```python
from build123d import *

# Parameters (mm, degrees)
BASE_BLOCK_DEPTH       = 42
TOP_BOSS_SKETCH_W      = 30
TOP_BOSS_SKETCH_H      = 30
TOP_BOSS_30X30_DEPTH   = 20
VERTICAL_BORE_SKETCH_R = 10
VERTICAL_BORE_DEPTH    = 98.693397935
CROSS_HOLE_SKETCH_R    = 6
CROSS_HOLE_DEPTH       = 75.759614766
ANGLED_POCKET_DEPTH    = 94.61448679
ARCH_CUTOUT_DEPTH      = 98.693397984
ARCH_CUTOUT_DEPTH_BACK = 98.693397984


with BuildPart() as part:
    # Base Block Profile Sketch → Base Block (new body)
    with BuildSketch(Plane.XY):
        Polygon((0, 0), (74, 0), (74, 28), (34, 28), (0, 20), align=None)
    extrude(amount=BASE_BLOCK_DEPTH)

    # Top Boss Sketch → Top Boss 30x30 (add)
    with BuildSketch(Plane(origin=(0, 28, 0), x_dir=(1, 0, 0), z_dir=(0, 1, 0))):
        with Locations((54, -21)):
            Rectangle(TOP_BOSS_SKETCH_W, TOP_BOSS_SKETCH_H)
    extrude(amount=TOP_BOSS_30X30_DEPTH)

    # Vertical Bore Sketch → Vertical Bore (cut, through all)
    with BuildSketch(Plane(origin=(0, 48, 0), x_dir=(1, 0, 0), z_dir=(0, 1, 0))):
        with Locations(Location((54, -21, 0), (0, 0, 180))):
            Circle(VERTICAL_BORE_SKETCH_R)
    extrude(amount=-VERTICAL_BORE_DEPTH, mode=Mode.SUBTRACT)

    # Cross Hole Sketch → Cross Hole (cut, through all)
    with BuildSketch(Plane.ZY.offset(-39)):
        with Locations((21, 38)):
            Circle(CROSS_HOLE_SKETCH_R)
    extrude(amount=-CROSS_HOLE_DEPTH, mode=Mode.SUBTRACT)

    # Angled Pocket Sketch → Angled Pocket (cut, through all)
    with BuildSketch(Plane(origin=(-4.459016393, 18.950819672, 0), x_dir=(0.973417168333576, 0.22903933372554744, 0), z_dir=(-0.22903933372554744, 0.973417168333576, 0))):
        Polygon((11.580786675, -21), (11.580786675, -15), (31.580786675, -15), (31.580786675, -27), (11.580786675, -27), align=None)
    extrude(amount=-ANGLED_POCKET_DEPTH, mode=Mode.SUBTRACT)

    # Arch Cutout Sketch → Arch Cutout (cut, two sides: drawn at the far end of the back side and taken through both)
    with BuildSketch(Plane.ZY.offset(-ARCH_CUTOUT_DEPTH_BACK)):
        with BuildLine():
            Line((36, -130.00000016), (36, 0))
            ThreePointArc((36, 0), (21, 15), (6, 0))
            Line((6, 0), (6, -130.00000016))
            Line((6, -130.00000016), (6, -390.00000048))
            Line((6, -390.00000048), (36, -390.00000048))
            Line((36, -390.00000048), (36, -130.00000016))
        make_face()
    extrude(amount=ARCH_CUTOUT_DEPTH + ARCH_CUTOUT_DEPTH_BACK, mode=Mode.SUBTRACT)


solid = part.part
```
Build history of the part. All positions in model axes, mm. A direction names the side the tool comes from. Round coordinates to 2 decimals unless told otherwise and drop trailing zeros. Order: outer loops, then holes, each group sorted by start corner. A loop starts at its lowest first (then second) coordinate and runs counter-clockwise, first axis right, second up. Notation, with made-up numbers: (48.5, -26) - (59.5, -26) arc R20 ccw to (59.5, -15) - close; hole circle Ø1 at (-17.5, 42.25). An arc over 180 degrees is marked (long way). Use a Markdown table: item, result.
1) Tool access for faces 1 (the face through (54, 38, 36)), 2 (the face through (69, 38, 28)), 3 (the face through (27.725, 20.053, 20.916)), 4 (the face through (7.725, 17.73, 20.916)): list every direction of +Z, -Z, +X, -X, +Y, -Y with a clear straight run to the whole face (end or side of a thin tool).
Recorded:
| item | result |
|---|---|
| face 1 | +Z, +X, -X, +Y |
| face 2 | +Z, -Z, +X, +Y |
| face 3 | -Y |
| face 4 | +Y |
2) Saw through at D-D on x = 65. Write the cut outline in (y, z).
Recorded:
| item | result |
|---|---|
| outline | (0, 0) - (28, 0) - (28, 6) - (48, 6) - (48, 36) - (28, 36) - (28, 42) - (0, 42) - (0, 36) arc R15 cw to (0, 6) - close; hole circle Ø12 at (38, 21) |
3) Wall check: L1, parallel to Y at x = 67, z = 21; L2, parallel to Z at x = 66.25, y = 38; L3, parallel to Z at x = 54, y = 27. Give the ranges that are in metal, low to high.
Recorded:
| item | result |
|---|---|
| L1 | y = 15 to 32, 44 to 48 |
| L2 | z = 6 to 15, 27 to 36 |
| L3 | z = 0 to 11, 31 to 42 |
4) Pull direction Z, two halves, no side cores. Call faces 5 (the face through (39, 38, 28)), 6 (the face through (41.67, 35.7, 26.54)), 7 (the face through (54, 38, 6)): pulls with the +Z half, pulls with the -Z half, needs draft (parallel to the pull), parting line crosses it, or undercut.
Recorded:
| item | result |
|---|---|
| face 5 | needs draft |
| face 6 | undercut |
| face 7 | pulls with the -Z half |
5) Saw through at B-B on y = 38. Write the cut outline in (x, z), and give its area (3 significant figures).
Recorded:
| item | result |
|---|---|
| outline | (39, 6) - (69, 6) - (69, 15) - (62, 15) arc R10 cw to (46, 15) - (39, 15) - close; (39, 27) - (46, 27) arc R10 cw to (62, 27) - (69, 27) - (69, 36) - (39, 36) - close |
| area | 451 mm² |
6) Saw through at A-A on x = 54. Write the cut outline in (y, z), and give its area (3 significant figures).
Recorded:
| item | result |
|---|---|
| outline | (0, 0) - (28, 0) - (28, 6) - (48, 6) - (48, 11) - (11.18, 11) arc R15 cw to (0, 6) - close; (0, 36) arc R15 cw to (11.18, 31) - (48, 31) - (48, 36) - (28, 36) - (28, 42) - (0, 42) - close |
| area | 739 mm² |
7) Saw through at C-C on z = 14. Write the cut outline in (x, y).
Recorded:
| item | result |
|---|---|
| outline | (0, 13.27) - (46.86, 13.27) - (46.86, 48) - (39, 48) - (39, 28) - (34, 28) - (0, 20) - close; (61.14, 13.27) - (74, 13.27) - (74, 28) - (69, 28) - (69, 48) - (61.14, 48) - close |
8) Flat gauge pins, fed straight in: pin 1 Ø7 at (y, z) = (38, 21) entering from +X; pin 2 Ø12 at (y, z) = (40.5, 35) entering from +X; pin 3 Ø2 at (x, z) = (40.5, 14) entering from -Y; pin 4 Ø15.5 at (y, z) = (38, 21) entering from -X. Where does each tip first touch, or does it go through?
Recorded:
| item | result |
|---|---|
| pin 1 | passes through |
| pin 2 | stops at x = 69 |
| pin 3 | stops at y = 12.69 |
| pin 4 | stops at x = 39 |
